Input: part model. Units: mm. Frame: model coordinates. A direction names the side the tool comes from. Coordinates: 2 decimals unless noted, no trailing zeros. Loops run counter-clockwise (first coordinate to the right, second up) from the corner with the lowest first, then second, coordinate; pieces in that order, holes last.
```python
from build123d import *

# Parameters (mm, degrees)
SKETCH1_W            = 370
SKETCH1_H            = 130
SKETCH1_R            = 12.5
BOSS_EXTRUDE1_DEPTH  = 10
M8_CLEARANCE_HOLE1_D = 10


with BuildPart() as part:
    # Sketch1 → Boss-Extrude1 (new body)
    with BuildSketch(Plane(origin=(0, 0, 0), x_dir=(-1, 0, 0), z_dir=(0, 0, -1))):
        with Locations((-185, 65)):
            Rectangle(SKETCH1_W, SKETCH1_H)
        with Locations(Location((-350, 20, 0), (0, 0, 180))):
            Circle(SKETCH1_R, mode=Mode.SUBTRACT)
        with Locations(Location((-20, 110, 0), (0, 0, 180))):
            Circle(SKETCH1_R, mode=Mode.SUBTRACT)
        with Locations(Location((-350, 110, 0), (0, 0, 180))):
            Circle(SKETCH1_R, mode=Mode.SUBTRACT)
        with Locations(Location((-20, 20, 0), (0, 0, 180))):
            Circle(SKETCH1_R, mode=Mode.SUBTRACT)
        with BuildLine():
            Line((-37.5, 52.5), (-332.5, 52.5))
            ThreePointArc((-332.5, 52.5), (-345, 65), (-332.5, 77.5))
            Line((-332.5, 77.5), (-37.5, 77.5))
            ThreePointArc((-37.5, 77.5), (-25, 65), (-37.5, 52.5))
        make_face(mode=Mode.SUBTRACT)
    extrude(amount=-BOSS_EXTRUDE1_DEPTH)

    # M8 Clearance Hole1 (through all)
    with Locations(Plane(origin=(0, 0, 0), x_dir=(-1, 0, 0), z_dir=(0, 0, -1))):
        with Locations((-245, 25), (-125, 25), (-125, 105), (-245, 105)):
            Hole(M8_CLEARANCE_HOLE1_D / 2)


solid = part.part
```
Item 1: Section query D-D (z = 6.25). Count the separate pieces of the cut face and the enclosed holes in it, then the cut area to 3 significant figures.
Result:
separate pieces: 1
enclosed holes: 9
area: 38,000 mm2
Item 2: Contact query for a flat-ended pin moving along its axis: P1, Ø15, axis at x = 350, y = 20, coming from the +Z side. Output: stop coordinate, or through.
Result:
P1: passes through
Item 3: Section query B-B (x = 46). Output: boundary loops of the cut face in (y, z).
Result:
outline: (0, 0) - (52.5, 0) - (52.5, 10) - (0, 10) - close; (77.5, 0) - (130, 0) - (130, 10) - (77.5, 10) - close
Item 4: Mould query, pull axis X, two halves, no side actions, for faces 3 (the face through (188, 80, 10)), 4 (the face through (0, 64, 5)), 5 (the face through (370, 64, 5)), 6 (the face through (25, 65, 5)). Classes: +X half, -X half, draft (parallel to the pull), parting line (faces both ways), or undercut.
Result:
face 3: draft
face 4: -X half
face 5: +X half
face 6: undercut
Item 5: Reachability of faces 1 (the face through (187, 77.5, 5)), 2 (the face through (188, 130, 5)) from +Z, -Z, +X, -X, +Y, -Y: full face, straight path, thin tool, end or side. Return the list, or none.
Result:
face 1: +Z, -Z
face 2: +Z, -Z, +X, -X, +Y
Item 6: Line query: L1, parallel to Y at x = 350, z = 3.5; L2, parallel to X at y = 64, z = 4.5; L3, parallel to Y at x = 125, z = 4.5. Output: solid intervals per line, ascending.
Result:
L1: y = 0 to 7.5, 32.5 to 97.5, 122.5 to 130
L2: x = 0 to 25.04, 344.96 to 370
L3: y = 0 to 20, 30 to 52.5, 77.5 to 100, 110 to 130
Item 7: Section query C-C (y = 105). Output: boundary loops of the cut face in (x, z), then the cut area to 3 significant figures.
Result:
outline: (0, 0) - (8.54, 0) - (8.54, 10) - (0, 10) - close; (31.46, 0) - (120, 0) - (120, 10) - (31.46, 10) - close; (130, 0) - (240, 0) - (240, 10) - (130, 10) - close; (250, 0) - (338.54, 0) - (338.54, 10) - (250, 10) - close; (361.46, 0) - (370, 0) - (370, 10) - (361.46, 10) - close
area: 3,040 mm2
Item 8: Section query A-A (x = 125). Output: boundary loops of the cut face in (y, z).
Result:
outline: (0, 0) - (20, 0) - (20, 10) - (0, 10) - close; (30, 0) - (52.5, 0) - (52.5, 10) - (30, 10) - close; (77.5, 0) - (100, 0) - (100, 10) - (77.5, 10) - close; (110, 0) - (130, 0) - (130, 10) - (110, 10) - close
